from build123d import *

# Parameters (mm, degrees)
SKETCH1_R           = 31.75
SKETCH1_R_2         = 2.667
BOSS_EXTRUDE1_DEPTH = 7.62
SKETCH2_R           = 6.604
CUT_EXTRUDE1_DEPTH  = 46.543269536
SKETCH_1_R          = 7.5
EXTRUDE_1_DEPTH     = 7.62
SKETCH_2_R          = 8
SKETCH_2_R_2        = 6.5
BOSS_EXTRUDE2_DEPTH = 50
SCALE1_SCALE        = 2
SKETCH3_R           = 6
CUT_EXTRUDE_1_DEPTH = 21
BOSS_EXTRUDE3_START = -15.24
SKETCH5_R           = 69.5
SKETCH5_R_2         = 63.5
BOSS_EXTRUDE3_DEPTH = 15.24


with BuildPart() as part:
    # Sketch1 → Boss-Extrude1 (new body)
    with BuildSketch(Plane(origin=(0, 0, 0), x_dir=(1, 0, 0), z_dir=(0, 1, 0))):
        with Locations(Location((0, 0, 0), (0, 0, 270))):
            Circle(SKETCH1_R)
        with Locations(Location((-15.24, 16.51, 0), (0, 0, 270))):
            Circle(SKETCH1_R_2, mode=Mode.SUBTRACT)
        with Locations(Location((15.24, 16.51, 0), (0, 0, 270))):
            Circle(SKETCH1_R_2, mode=Mode.SUBTRACT)
        with Locations(Location((15.24, -16.51, 0), (0, 0, 270))):
            Circle(SKETCH1_R_2, mode=Mode.SUBTRACT)
        with Locations(Location((-15.24, -16.51, 0), (0, 0, 270))):
            Circle(SKETCH1_R_2, mode=Mode.SUBTRACT)
    extrude(amount=-BOSS_EXTRUDE1_DEPTH)

    # Sketch2 → Cut-Extrude1 (cut, through all)
    with BuildSketch(Plane(origin=(0, 0, 0), x_dir=(1, 0, 0), z_dir=(0, 1, 0))):
        with Locations(Location((0, 0, 0), (0, 0, 270))):
            Circle(SKETCH2_R)
    extrude(amount=-CUT_EXTRUDE1_DEPTH, mode=Mode.SUBTRACT)

    # 草图1 → 凸台-拉伸1 (add)
    with BuildSketch(Plane.XZ.offset(7.62)):
        Circle(SKETCH_1_R)
    extrude(amount=-EXTRUDE_1_DEPTH)

    # 草图2 → Boss-Extrude2 (add)
    with BuildSketch(Plane(origin=(0, 0, 0), x_dir=(1, 0, 0), z_dir=(0, 1, 0))):
        with Locations(Location((0, 0, 0), (0, 0, 270))):
            Circle(SKETCH_2_R)
        with Locations(Location((0, 0, 0), (0, 0, 270))):
            Circle(SKETCH_2_R_2, mode=Mode.SUBTRACT)
    extrude(amount=BOSS_EXTRUDE2_DEPTH)


with BuildPart() as part_1:
    # Scale1: scaled about (0, 0, 0)
    add(part.part.scale(SCALE1_SCALE))

    # Sketch3 → 切除-拉伸1 (cut)
    with BuildSketch(Plane(origin=(0, 0, 0), x_dir=(1, 0, 0), z_dir=(0, 1, 0))):
        with Locations(Location((56.568542495, 0, 0), (0, 0, 270))):
            Circle(SKETCH3_R)
        with Locations(Location((0, -56.568542495, 0), (0, 0, 270))):
            Circle(SKETCH3_R)
        with Locations(Location((-56.568542495, 0, 0), (0, 0, 270))):
            Circle(SKETCH3_R)
        with Locations(Location((0, 56.568542495, 0), (0, 0, 270))):
            Circle(SKETCH3_R)
    extrude(amount=-CUT_EXTRUDE_1_DEPTH, mode=Mode.SUBTRACT)

    # Sketch5 → Boss-Extrude3 (add)
    with BuildSketch(Plane.XZ.offset(15.24).offset(BOSS_EXTRUDE3_START)):
        with Locations(Location((0, 0, 0), (0, 0, 270))):
            Circle(SKETCH5_R)
        Circle(SKETCH5_R_2, mode=Mode.SUBTRACT)
    extrude(amount=BOSS_EXTRUDE3_DEPTH)


solid = part_1.part
Model file for the job. Use its own axes, mm. A direction names the side the tool comes from. Coordinates: 2 decimals unless noted, no trailing zeros. Order: outer loops, then holes, each group sorted by start corner. A loop starts at its lowest first (then second) coordinate and runs counter-clockwise, first axis right, second up. Notation, with made-up numbers: M 73.5,-19 L 124.5,-19 A24 ccw 124.5,17 Z; hole C 58.25,46.5 d7. An arc over 180 degrees is marked long. Return JSON: item names as keys, results as strings.
1. Saw through at A-A (x = 0). Give the cut face in (y, z).
Ans:
{"outline": "M -15.24,-69.5 L 0,-69.5 L 0,-62.57 L -15.24,-62.57 Z; M -15.24,-50.57 L 0,-50.57 L 0,-16 L 100,-16 L 100,-13 L 0,-13 L 0,13 L 100,13 L 100,16 L 0,16 L 0,50.57 L -15.24,50.57 Z; M -15.24,62.57 L 0,62.57 L 0,69.5 L -15.24,69.5 Z"}
2. Saw through at B-B (y = -2.5). Give the number of separate pieces and of enclosed holes in the cut face, and give its area (3 significant figures).
Ans:
{"separate pieces": "1", "enclosed holes": "8", "area": "14,400 mm^2"}
3. Drill centre lines: probe 1 along X at (y, z) = (-6, 0); probe 2 along X at (y, z) = (62, 0); probe 3 along Z at (x, y) = (30, -9). Where is each one in solid material? Low to high.
Ans:
{"probe 1": "-69.5 to -62.57, -50.57 to 50.57, 62.57 to 69.5", "probe 2": "-16 to -13, 13 to 16", "probe 3": "-62.69 to -38.33, -27.71 to 27.71, 38.33 to 62.69"}
4. Saw through at D-D (x = 59.5). Give the cut face in (y, z), and give its area (3 significant figures).
Ans:
{"outline": "M -15.24,-35.92 L 0,-35.92 L 0,-5.24 L -15.24,-5.24 Z; M -15.24,5.24 L 0,5.24 L 0,35.92 L -15.24,35.92 Z", "area": "935 mm^2"}
5. Saw through at C-C (z = -33.02). Give the cut face in (x, y), and give its area (3 significant figures).
Ans:
{"outline": "M -61.15,-15.24 L -35.81,-15.24 L -35.81,0 L -61.15,0 Z; M -25.15,-15.24 L 25.15,-15.24 L 25.15,0 L -25.15,0 Z; M 35.81,-15.24 L 61.15,-15.24 L 61.15,0 L 35.81,0 Z", "area": "1,540 mm^2"}
6. Flat gauge pins, fed straight in: pin 1 (6 mm diameter, centred on y = 63, z = 6, fed in from +X); pin 2 (2 mm diameter, centred on y = 35, z = -9.5, fed in from -X); pin 3 (1.5 mm diameter, centred on x = 1.5, z = 18, fed in from +Y). Where does each tip first touch, or does it go through?
Ans:
{"pin 1": "x = 15.72", "pin 2": "x = -13.56", "pin 3": "y = 0"}
7. Pull direction Z, two halves, no side cores. Call faces 1 (the face through (16.4, 0, 1)), 2 (the face through (-30.25, -7.51, -38.35)), 3 (the face through (-2.298, -7.513, -51.026)), 4 (the face through (68.91, -7.51, 9.05)): +Z half, -Z half, draft (parallel to the pull), parting line (faces both ways), or undercut.
Ans:
{"face 1": "draft", "face 2": "undercut", "face 3": "undercut", "face 4": "parting line"}
8. Tool access for faces 5 (the face through (0, 0, 0)), 6 (the face through (-33.73, -7.51, 28.79)): list every direction of +Z, -Z, +X, -X, +Y, -Y with a clear straight run to the whole face (end or side of a thin tool).
Ans:
{"face 5": "+Y", "face 6": "+Y, -Y"}
